Design review of the part built by this model. Coordinates are the model's own, in mm. A direction names the side the tool comes from. Give positions to 0.01 mm unless a question says otherwise; leave off trailing zeros. Order: outer loops, then holes, each group sorted by start corner. A loop starts at its lowest first (then second) coordinate and runs counter-clockwise, first axis right, second up. Notation, with made-up numbers: M 49,53.5 L 106,53.5 A28 cw 106,72.5 Z; hole C 35.25,-10.75 d4. An arc over 180 degrees is marked long. Put each result on its own line as item: value. Start each with the question number.
from build123d import *

# Parameters (mm, degrees)
SKETCH_1_R      = 15
EXTRUDE_1_DEPTH = 5
EXTRUDE_2_DEPTH = 5
M3X0_5_1_D      = 2.5
M3X0_5_1_DEPTH  = 7.5
M3X0_5_1_TIP    = 0.751075774


with BuildPart() as part:
    # 草图1 → 凸台-拉伸1 (new, symmetric)
    with BuildSketch(Plane.XY):
        Circle(SKETCH_1_R)
        with BuildLine():
            Line((11, 1.802775638), (11, -1.802775638))
            ThreePointArc((11, -1.802775638), (4.5, 0), (11, 1.802775638))
        make_face(mode=Mode.SUBTRACT)
    extrude(amount=EXTRUDE_1_DEPTH, both=True)

    # 草图4 → 旋转1 (revolve)
    with BuildSketch(Plane(origin=(0, 0, 0), x_dir=(1, 0, 0), z_dir=(0, 1, 0))):
        with BuildLine():
            Line((18.2, 5), (15, 5))
            Line((15, 5), (15, 0))
            ThreePointArc((15, 0), (15.9372583, 2.2627417), (18.2, 3.2))
            Line((18.2, 3.2), (18.2, 5))
        make_face()
        with BuildLine():
            ThreePointArc((18.2, -3.2), (15.9372583, -2.2627417), (15, 0))
            Line((15, 0), (15, -5))
            Line((15, -5), (18.2, -5))
            Line((18.2, -5), (18.2, -3.2))
        make_face()
    revolve(axis=Axis((0, 0, 0), (0, 0, -1)))

    # 草图5 → 凸台-拉伸2 (add)
    with BuildSketch(Plane.XY.offset(-5)):
        with BuildLine():
            Line((14, -2.5), (14, 2.5))
            ThreePointArc((14, 2.5), (1.5, 0), (14, -2.5))
        make_face()
        with BuildLine():
            Line((11, -1.802775638), (11, 1.802775638))
            ThreePointArc((11, 1.802775638), (4.5, 0), (11, -1.802775638))
        make_face(mode=Mode.SUBTRACT)
    extrude(amount=-EXTRUDE_2_DEPTH)

    # M3x0.5 螺纹孔1
    with Locations(Plane(origin=(14, 0, -7.5), x_dir=(0, 0, 1), z_dir=(1, 0, 0))):
        with Locations((0, 0)):
            Hole(M3X0_5_1_D / 2, depth=M3X0_5_1_DEPTH)
            with Locations((0, 0, -(M3X0_5_1_DEPTH + M3X0_5_1_TIP / 2))):  # 118° drill point
                Cone(0, M3X0_5_1_D / 2, M3X0_5_1_TIP, mode=Mode.SUBTRACT)


solid = part.part
1. Machinability: for faces 1 (the cylindrical face through (1.505, 0.25, -7.465)), 2 (the flat face through (14, -1, -6)), 3 (the cylindrical face through (12.48, -0.05, -6.25)), 4 (the flat face through (0, 0, 5)), which of the approach directions +Z, -Z, +X, -X, +Y, -Y give a long, thin tool a straight path to every point of the face, cutting with its end or side? Answer none if there is none.
2. Consider section B-B on z = -2.25. Give the boundary of the cut face in (x, y), then the cut area to 3 significant figures.
3. The part is to be moulded in two halves that separate along Y. For faces 5 (the flat face through (11, 0, -2)), 6 (the flat face through (10.4, -2.8, -10)), 7 (the cylindrical face through (-3.945, 17.767, 4.087)), say which applies: +Y half, -Y half, draft (parallel to the pull), parting line (faces both ways), or undercut.
4. Insertion check: pin 1 (1.8 mm diameter, centred on y = 1, z = -1, fed in from -X); pin 2 (4 mm diameter, centred on y = -14, z = 1.5, fed in from +X); pin 3 (2.5 mm diameter, centred on y = -1, z = -8, fed in from +X); pin 4 (5.5 mm diameter, centred on x = 8, y = 0, fed in from +Z). Each pin has a flat end and moves straight along its axis. Give the tip position at first contact, or say it passes through.
5. To check wall thickness, follow probe 1 along Y at (x, z) = (8, -9); probe 2 along Z at (x, y) = (0, 4); probe 3 along X at (y, z) = (1, 1). State the ranges of each line that lie inside material, in increasing order.
6. Consider section A-A on z = -7.5. Give the boundary of the cut face in (x, y), then the cut area to 3 significant figures.
Returned:
1. face 1: -Z
1. face 2: -Z, +X, +Y, -Y
1. face 3: +X
1. face 4: +Z, +X, -X, +Y, -Y
2. outline: C 0,0 d31.85; hole M 11,-1.8 L 11,1.8 A3.5 ccw long Z
2. area: 759 mm2
3. face 5: undercut
3. face 6: draft
3. face 7: parting line
4. pin 1: stops at x = -15.6
4. pin 2: stops at x = 12.79
4. pin 3: stops at x = 14
4. pin 4: passes through
5. probe 1: y = -6.5 to -3.5, 3.5 to 6.5
5. probe 2: z = -5 to 5
5. probe 3: x = -15.13 to 4.65, 11 to 15.13
6. outline: M 11,-1.8 A3.5 cw long 11,1.8 L 11,1.25 L 14,1.25 L 14,2.5 A6.5 ccw long 14,-2.5 L 14,-1.25 L 11,-1.25 Z
6. area: 86.3 mm2
